from build123d import *

# Parameters (mm, degrees)
SKETCH1_R           = 4
BOSS_EXTRUDE1_DEPTH = 45.65
SKETCH2_R           = 5
BOSS_EXTRUDE2_DEPTH = 1
SKETCH3_R           = 4
BOSS_EXTRUDE3_DEPTH = 42.74
CUT_EXTRUDE1_DEPTH  = 1.8


with BuildPart() as part:
    # Sketch1 → Boss-Extrude1 (new body)
    with BuildSketch(Plane.XY):
        Circle(SKETCH1_R)
    extrude(amount=BOSS_EXTRUDE1_DEPTH)

    # Sketch2 → Boss-Extrude2 (add)
    with BuildSketch(Plane.XY.offset(45.65)):
        Circle(SKETCH2_R)
    extrude(amount=BOSS_EXTRUDE2_DEPTH)

    # Sketch3 → Boss-Extrude3 (add)
    with BuildSketch(Plane.XY.offset(46.65)):
        Circle(SKETCH3_R)
    extrude(amount=BOSS_EXTRUDE3_DEPTH)

    # Sketch4 → Cut-Extrude1 (cut)
    with BuildSketch(Plane(origin=(0, 4, 0), x_dir=(1, 0, 0), z_dir=(0, 1, 0))):
        with BuildLine():
            Line((1.5, -3.5), (1.5, -8.5))
            ThreePointArc((1.5, -8.5), (0, -10), (-1.5, -8.5))
            Line((-1.5, -8.5), (-1.5, -3.5))
            ThreePointArc((-1.5, -3.5), (0, -2), (1.5, -3.5))
        make_face()
        with BuildLine():
            Line((1.5, -39.15), (1.5, -44.15))
            ThreePointArc((1.5, -44.15), (0, -45.65), (-1.5, -44.15))
            Line((-1.5, -44.15), (-1.5, -39.15))
            ThreePointArc((-1.5, -39.15), (0, -37.65), (1.5, -39.15))
        make_face()
        with BuildLine():
            Line((1.5, -80.89), (1.5, -85.89))
            ThreePointArc((1.5, -85.89), (0, -87.39), (-1.5, -85.89))
            Line((-1.5, -85.89), (-1.5, -80.89))
            ThreePointArc((-1.5, -80.89), (0, -79.39), (1.5, -80.89))
        make_face()
    extrude(amount=-CUT_EXTRUDE1_DEPTH, mode=Mode.SUBTRACT)


solid = part.part
Can you work these out from the model? Positions are in its coordinate system, mm. A direction names the side the tool comes from. Coordinates: 2 decimals unless noted, no trailing zeros. Loops run counter-clockwise (first coordinate to the right, second up) from the corner with the lowest first, then second, coordinate; pieces in that order, holes last. Notation, with made-up numbers: M 58.25,-38 L 115.25,-38 A9 ccw 115.25,-27 Z; hole C 60.25,75 d3. An arc over 180 degrees is marked long. Return JSON: item names as keys, results as strings. Group by question number.
Item 1: If I drill on L1, parallel to Z at x = -0.5, y = 3.5; L2, parallel to Z at x = 4, y = 1; L3, parallel to X at y = 0.25, z = 40.5, over which ranges is the centre line in solid material (lowest first)? Write a range as from..to.
Item 2: Thinking about a two-plate mould opening in Z: for faces 4 (the flat face through (0, 0, 89.39)), 5 (the flat face through (0, 0, 0)), 6 (the flat face through (1.5, 3, 42)), which applies, released by +Z, released by -Z, zero draft, split by the parting line, or undercut?
Item 3: Imagine slicing it at B-B (z = 36.5). Please give me the cut outline in (x, y), and give its area (3 significant figures).
Item 4: On a 3-axis mill with a long thin cutter (end or side, diameter ignored), from which of +Z, -Z, +X, -X, +Y, -Y can I reach the whole of each face in a straight line? I mean faces 1 (the cylindrical face through (0.03, 3.11, 87.39)), 2 (the cylindrical face through (-0.867, -3.905, 22.505)), 3 (the cylindrical face through (-0.867, -3.905, 67.721)). Say none if no direction works.
Item 5: I'm going to push flat-ended pins straight in: pin 1 Ø4 at (x, y) = (-3.5, 2.5) entering from -Z; pin 2 Ø4 at (x, z) = (-0.5, 32) entering from -Y; pin 3 Ø1.7 at (y, z) = (2.5, 83.5) entering from -X; pin 4 Ø3 at (x, z) = (-0.5, 66.5) entering from +Y. Where does each tip first touch, or does it pass through?
Item 6: Imagine slicing it at A-A (y = -1). Please give me the cut outline in (x, z).
Verdict:
{
 "1": {"L1": "z = 0..2.09, 9.91..37.74, 45.56..79.48, 87.3..89.39", "L2": "z = 45.65..46.65", "L3": "x = -3.99..3.99"},
 "2": {"face 4": "released by +Z", "face 5": "released by -Z", "face 6": "undercut"},
 "3": {"outline": "C 0,0 d8", "area": "50.3 mm^2"},
 "4": {"face 1": "+Y", "face 2": "-Z", "face 3": "+Z"},
 "5": {"pin 1": "stops at z = 0", "pin 2": "stops at y = -4", "pin 3": "stops at x = -3.64", "pin 4": "stops at y = 4"},
 "6": {"outline": "M -4.9,45.65 L -3.87,45.65 L -3.87,0 L 3.87,0 L 3.87,45.65 L 4.9,45.65 L 4.9,46.65 L 3.87,46.65 L 3.87,89.39 L -3.87,89.39 L -3.87,46.65 L -4.9,46.65 Z"}
}
